Can you work these out from the model? Positions are in its coordinate system, mm. Coordinates: 2 decimals unless noted, no trailing zeros. Loops run counter-clockwise (first coordinate to the right, second up) from the corner with the lowest first, then second, coordinate; pieces in that order, holes last.
```python
from build123d import *

# Parameters (mm, degrees)
SKETCH1_W           = 850
SKETCH1_H           = 120
BOSS_EXTRUDE1_DEPTH = 20
CHAMFER1_SIZE       = 15


with BuildPart() as part:
    # Sketch1 → Boss-Extrude1 (new, symmetric)
    with BuildSketch(Plane.XY):
        Rectangle(SKETCH1_W, SKETCH1_H)
    extrude(amount=BOSS_EXTRUDE1_DEPTH, both=True)

    # Chamfer1
    chamfer1_edges = [part.edges().sort_by_distance(p)[0] for p in [
        (0, 60, 20),
        (0, 60, -20),
    ]]
    chamfer(chamfer1_edges, length=CHAMFER1_SIZE)


solid = part.part
```
(1) I'm going to push flat-ended pins straight in: pin 1 (2 mm diameter, centred on x = 317, z = -7.5, fed in from +Y); pin 2 (12 mm diameter, centred on x = -339, z = 11.5, fed in from +Y). Where does each tip first touch, or does it pass through?
Check values:
pin 1: stops at y = 58.5
pin 2: stops at y = 59.5
(2) I want a section at A-A on x = 354. Write out the boundary of the cut face in (y, z).
Check values:
outline: (-60, -20) - (45, -20) - (60, -5) - (60, 5) - (45, 20) - (-60, 20) - close
(3) If I drill on probe 1 along Y at (x, z) = (-193, 16.5); probe 2 along Y at (x, z) = (-65.5, -14.5), over which ranges is the centre line in solid material (lowest first)?
Check values:
probe 1: y = -60 to 48.5
probe 2: y = -60 to 50.5
